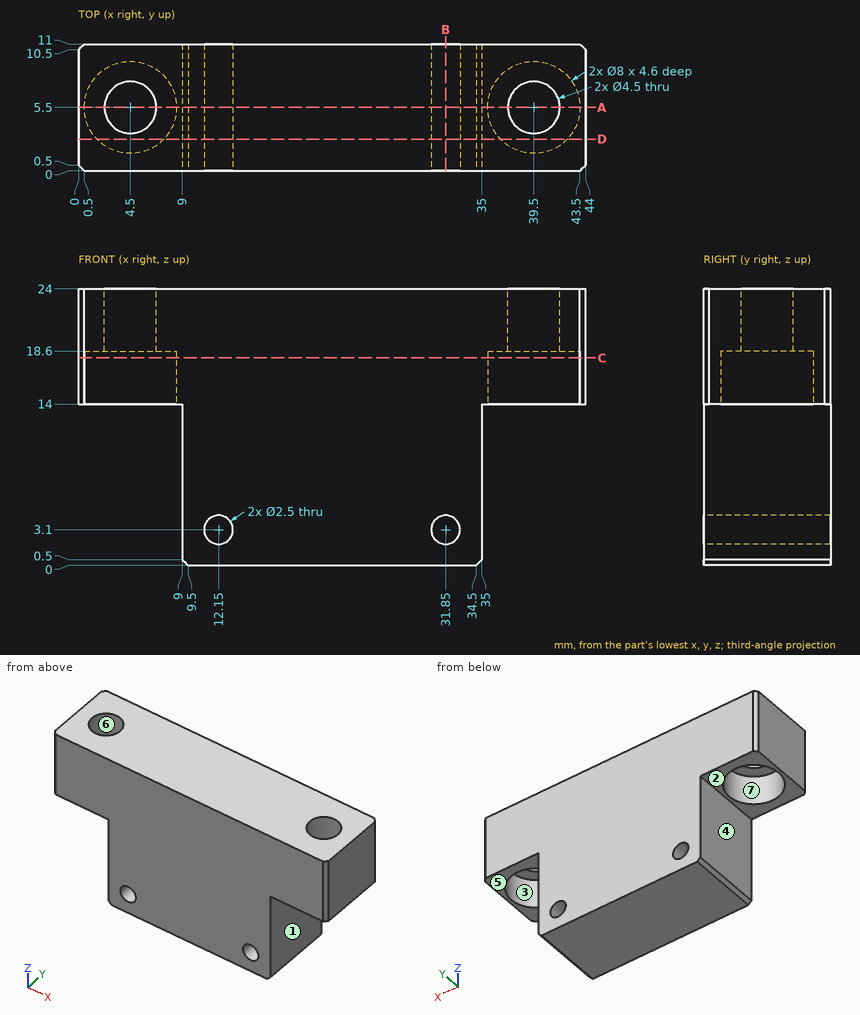
Design review of the part shown in the three views and the two pictorial views. Dimensions are in mm from the part's minimum x, y and z. A direction names the side the tool comes from. Give positions to 0.01 mm unless a question says otherwise; leave off trailing zeros. Write each loop counter-clockwise with the first axis right and the second up, starting at its lowest first coordinate (ties: lowest second). Pieces come first, ordered by that corner, then holes. Notation, with made-up numbers: M 18.25,78.25 L 24.25,78.25 A15 cw 24.25,97.25 Z; hole C 8.25,48 d9. An arc over 180 degrees is marked long. One line per item, written item: value.
1) For line 1 (X direction, y = 5.25, z = 14.5); line 2 (X direction, y = 9, z = 15.75); line 3 (Z direction, x = 31.85, y = 5), list the stretches that pass through material, from the lowest coordinate up. Write a range as from..to.
Results are:
line 1: x = 0..0.51, 8.49..35.51, 43.49..44
line 2: x = 0..2.56, 6.44..37.56, 41.44..44
line 3: z = 0..1.85, 4.35..24
2) Take a section at A-A, the plane y = 5.5. Write out the cut boundary in (x, z).
Results are:
outline: M 0,14 L 0.5,14 L 0.5,18.6 L 2.25,18.6 L 2.25,24 L 0,24 Z; M 6.75,18.6 L 8.5,18.6 L 8.5,14 L 9,14 L 9,0.5 L 9.5,0 L 34.5,0 L 35,0.5 L 35,14 L 35.5,14 L 35.5,18.6 L 37.25,18.6 L 37.25,24 L 6.75,24 Z; M 41.75,18.6 L 43.5,18.6 L 43.5,14 L 44,14 L 44,24 L 41.75,24 Z; hole C 12.15,3.1 d2.5; hole C 31.85,3.1 d2.5
3) Take a section at B-B, the plane x = 31.85. Write out the cut boundary in (y, z).
Results are:
outline: M 0,0 L 11,0 L 11,1.85 L 0,1.85 Z; M 0,4.35 L 11,4.35 L 11,24 L 0,24 Z
4) For the marked faces 1, 2 and 3, list the 3-axis set-ups (+Z, -Z, +X, -X, +Y, -Y) from which the entire face can be reached by the end or side of a thin tool; tool diameter is ignored.
Results are:
face 1: -Z, +X, +Y, -Y
face 2: -Z, -X, +Y, -Y
face 3: -Z
5) Take a section at D-D, the plane y = 2.75. Write out the cut boundary in (x, z).
Results are:
outline: M 0,14 L 1.6,14 L 1.6,18.6 L 7.4,18.6 L 7.4,14 L 9,14 L 9,0.5 L 9.5,0 L 34.5,0 L 35,0.5 L 35,14 L 36.6,14 L 36.6,18.6 L 42.4,18.6 L 42.4,14 L 44,14 L 44,24 L 0,24 Z; hole C 12.15,3.1 d2.5; hole C 31.85,3.1 d2.5
6) For P1, Ø4, axis at x = 4.5, y = 5.5, coming from the +Z side; P2, Ø6.5, axis at x = 4.5, y = 5, coming from the -Z side; P3, Ø3.5, axis at y = 4.5, z = 10, coming from the +X side; P4, Ø4, axis at y = 7.5, z = 9, coming from the -X side, all flat-tipped, find the tip position at first contact; note any pin that passes through.
Results are:
P1: passes through
P2: stops at z = 18.6
P3: stops at x = 35
P4: stops at x = 9
7) Take a section at C-C, the plane z = 18. Write out the cut boundary in (x, y).
Results are:
outline: M 0,0.5 L 0.5,0 L 43.5,0 L 44,0.5 L 44,10.5 L 43.5,11 L 0.5,11 L 0,10.5 Z; hole C 4.5,5.5 d8; hole C 39.5,5.5 d8
8) The part is to be moulded in two halves that separate along X. For the marked faces 4, 5, 6 and 7, say which applies: +X half, -X half, draft (parallel to the pull), parting line (faces both ways), or undercut.
Results are:
face 4: -X half
face 5: draft
face 6: undercut
face 7: undercut
